For this review, use the dimensioned drawing (mm, ordinates from the lowest corner) and the shaded views. Give positions to 0.01 mm unless a question says otherwise; leave off trailing zeros. Order: outer loops, then holes, each group sorted by start corner. A loop starts at its lowest first (then second) coordinate and runs counter-clockwise, first axis right, second up. Notation, with made-up numbers: (85, 5) - (115, 5) arc R35 cw to (115, 42) - close; hole circle Ø10 at (67.5, -15.5). An arc over 180 degrees is marked (long way). Use a Markdown table: item, result. Add a question column.
1) We need section A-A on z = 1.1. Write out the cut boundary in (x, y).
2) We need section B-B on x = 61.5. Write out the cut boundary in (y, z).
3) We need section C-C on y = 222. Write out the cut boundary in (x, z), then the cut area to 3 significant figures.
4) Wall thickness on L1, parallel to Y at x = 164.5, z = 4.55; L2, parallel to X at y = 106.5, z = 0.4; L3, parallel to Y at x = 247, z = 2.5: over which ranges is each line inside the solid? List them lowest first.
5) Clearance check with a flat-ended pin moving along its axis: P1, Ø1.5, axis at y = 138, z = 0.5, coming from the -X side. State where the tip first meets the part, or that it passes through.
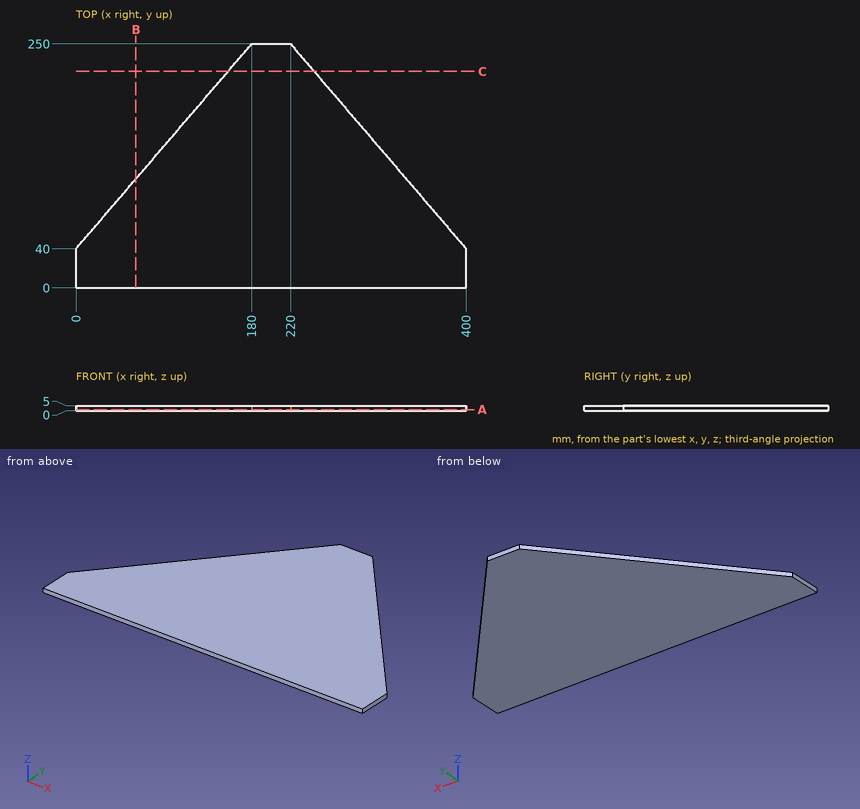
Checked values:
| question | item | result |
|---|---|---|
| 1 | outline | (0, 0) - (400, 0) - (400, 40) - (220, 250) - (180, 250) - (0, 40) - close |
| 2 | outline | (0, 0) - (111.75, 0) - (111.75, 5) - (0, 5) - close |
| 3 | outline | (156, 0) - (244, 0) - (244, 5) - (156, 5) - close |
| 3 | area | 440 mm² |
| 4 | L1 | 0 to 231.92 |
| 4 | L2 | 57 to 343 |
| 4 | L3 | 0 to 218.5 |
| 5 | P1 | x = 83.36 |
